```python
from build123d import *

# Parameters (mm, degrees)
SKETCH1_W             = 120
SKETCH1_H             = 9
BOSS_EXTRUDE1_DEPTH   = 5
M3_TAPPED_HOLE1_D     = 2.5
M3_TAPPED_HOLE1_DEPTH = 8.5
FILLET1_R             = 2
SKETCH4_W             = 35
SKETCH4_H             = 4.5
CUT_EXTRUDE1_DEPTH    = 121.440856855
FILLET2_R             = 2
SKETCH5_W             = 24
SKETCH5_H             = 9
CUT_EXTRUDE2_DEPTH    = 1.5


with BuildPart() as part:
    # Sketch1 → Boss-Extrude1 (new body)
    with BuildSketch(Plane(origin=(0, 0, 0), x_dir=(1, 0, 0), z_dir=(0, 1, 0))):
        with Locations((60, 4.5)):
            Rectangle(SKETCH1_W, SKETCH1_H)
    extrude(amount=BOSS_EXTRUDE1_DEPTH)

    # M3 Tapped Hole1
    with Locations(Plane(origin=(0, 5, 0), x_dir=(-1, 0, 0), z_dir=(0, 1, 0))):
        with Locations((-30, -4), (-110, -4)):
            Hole(M3_TAPPED_HOLE1_D / 2, depth=M3_TAPPED_HOLE1_DEPTH)

    # Fillet1
    fillet1_edges = [part.edges().sort_by_distance(p)[0] for p in [
        (0, 2.5, -9),
        (120, 2.5, -9),
    ]]
    fillet(fillet1_edges, radius=FILLET1_R)

    # Sketch4 → Cut-Extrude1 (cut, through all)
    with BuildSketch(Plane(origin=(0, 5, 0), x_dir=(-1, 0, 0), z_dir=(0, 1, 0))):
        with Locations((-77, -6.75)):
            Rectangle(SKETCH4_W, SKETCH4_H)
    extrude(amount=-CUT_EXTRUDE1_DEPTH, mode=Mode.SUBTRACT)

    # Fillet2
    fillet2_edges = [part.edges().sort_by_distance(p)[0] for p in [
        (94.5, 2.5, -9),
        (59.5, 2.5, -9),
    ]]
    fillet(fillet2_edges, radius=FILLET2_R)

    # Sketch5 → Cut-Extrude2 (cut)
    with BuildSketch(Plane.XZ):
        with Locations((77, -4.5)):
            Rectangle(SKETCH5_W, SKETCH5_H)
    extrude(amount=-CUT_EXTRUDE2_DEPTH, mode=Mode.SUBTRACT)


solid = part.part
```
Input: part model. Units: mm. Frame: model coordinates. A direction names the side the tool comes from. Round coordinates to 2 decimals unless told otherwise and drop trailing zeros. Loops run counter-clockwise (first coordinate to the right, second up) from the corner with the lowest first, then second, coordinate; pieces in that order, holes last.
1) Section query B-B on z = -8. Return the cut outline in (x, y).
Ans:
outline: (0.27, 0) - (59.23, 0) - (59.23, 5) - (0.27, 5) - close; (94.77, 0) - (119.73, 0) - (119.73, 5) - (94.77, 5) - close
2) Section query D-D on x = 80. Return the cut outline in (y, z), plus the area to 4 significant figures.
Ans:
outline: (1.5, -4.5) - (5, -4.5) - (5, 0) - (1.5, 0) - close
area: 15.75 mm2
3) Section query A-A on x = 110. Return the cut outline in (y, z), plus the area to 3 significant figures.
Ans:
outline: (0, -9) - (5, -9) - (5, -5.25) - (0, -5.25) - close; (0, -2.75) - (5, -2.75) - (5, 0) - (0, 0) - close
area: 32.5 mm2
4) Pull-direction query (X, two-part tool) for faces 1 (the flat face through (77, 1.5, -2)), 2 (the flat face through (0, 2, -3)), 3 (the flat face through (77, 3, -4.5)), 4 (the flat face through (120, 2, -3)); classes: released by +X, released by -X, zero draft, split by the parting line, or undercut.
Ans:
face 1: undercut
face 2: released by -X
face 3: undercut
face 4: released by +X
5) Section query C-C on y = 2.8. Return the cut outline in (x, z), plus the area to 3 significant figures.
Ans:
outline: (0, -7) arc R2 ccw to (2, -9) - (57.5, -9) arc R2 ccw to (59.5, -7) - (59.5, -4.5) - (94.5, -4.5) - (94.5, -7) arc R2 ccw to (96.5, -9) - (118, -9) arc R2 ccw to (120, -7) - (120, 0) - (0, 0) - close; hole circle Ø2.5 at (30, -4); hole circle Ø2.5 at (110, -4)
area: 909 mm2
6) Material intervals for line 1 (Z direction, x = 110, y = 2.6); line 2 (X direction, y = 2.7, z = -3); line 3 (X direction, y = 3.8, z = -6), sorted ascending.
Ans:
line 1: z = -9 to -5.25, -2.75 to 0
line 2: x = 0 to 29.25, 30.75 to 109.25, 110.75 to 120
line 3: x = 0 to 59.5, 94.5 to 120
7) Pin query (flat end, axial travel): pin 1 (2 mm diameter, centred on x = 81, z = -2.5, fed in from -Y). Return the tip coordinate at first contact, or that it passes through.
Ans:
pin 1: stops at y = 1.5
8) Set-up query: faces 5 (the cylindrical face through (0.57, 2.54, -8.4)), 6 (the cylindrical face through (95.07, 2.46, -8.4)). Return all of +Z, -Z, +X, -X, +Y, -Y with unobstructed straight access to the full face (end or side cutting, diameter ignored); none if empty.
Ans:
face 5: -Z, -X, +Y, -Y
face 6: -Z, +Y, -Y
